Model file for the job. Use its own axes, mm. A direction names the side the tool comes from. Round coordinates to 2 decimals unless told otherwise and drop trailing zeros. Write each loop counter-clockwise with the first axis right and the second up, starting at its lowest first coordinate (ties: lowest second). Pieces come first, ordered by that corner, then holes. Notation, with made-up numbers: (-24, 53.5) - (12, 53.5) arc R7 ccw to (12, 66.5) - close; hole circle Ø7 at (20, -9). An arc over 180 degrees is marked (long way). One line per item, written item: value.
from build123d import *

# Parameters (mm, degrees)
BOSS_EXTRUDE1_DEPTH = 350


with BuildPart() as part:
    # Sketch1 → Boss-Extrude1 (new body)
    with BuildSketch(Plane.XY):
        with BuildLine():
            Line((0, 0), (30, 0))
            Line((30, 0), (30, 1))
            ThreePointArc((30, 1), (29.414213562, 2.414213562), (28, 3))
            Line((28, 3), (5, 3))
            ThreePointArc((5, 3), (3.585786438, 3.585786438), (3, 5))
            Line((3, 5), (3, 28))
            ThreePointArc((3, 28), (2.414213562, 29.414213562), (1, 30))
            Line((1, 30), (0, 30))
            Line((0, 30), (0, 0))
        make_face()
    extrude(amount=BOSS_EXTRUDE1_DEPTH)


solid = part.part
1. Drop flat-ended pins along their axis: pin 1 (12 mm diameter, centred on y = 23, z = 100, fed in from +X); pin 2 (12 mm diameter, centred on x = 10, z = 165, fed in from -Y); pin 3 (3 mm diameter, centred on y = 3, z = 238.5, fed in from +X); pin 4 (7 mm diameter, centred on x = 12, z = 141, fed in from +Y). Give the stop position or say it passes through.
Report:
pin 1: x = 3
pin 2: y = 0
pin 3: x = 29.94
pin 4: y = 3
2. Wall check: probe 1 along X at (y, z) = (14, 96); probe 2 along Y at (x, z) = (4.5, 296.5). Give the ranges that are in metal, low to high. Write a range as [from, to].
Report:
probe 1: [0, 3]
probe 2: [0, 3.06]
3. Band-saw the part on A-A on z = 243.5. Write the cut outline in (x, y).
Report:
outline: (0, 0) - (30, 0) - (30, 1) arc R2 ccw to (28, 3) - (5, 3) arc R2 cw to (3, 5) - (3, 28) arc R2 ccw to (1, 30) - (0, 30) - close
4. Band-saw the part on B-B on y = 15. Write the cut outline in (x, z).
Report:
outline: (0, 0) - (3, 0) - (3, 350) - (0, 350) - close
5. Tool access for faces 1 (the face through (17, 3, 173)), 2 (the face through (2.7, 9.5, 0)): list every direction of +Z, -Z, +X, -X, +Y, -Y with a clear straight run to the whole face (end or side of a thin tool).
Report:
face 1: +Z, -Z, +X, +Y
face 2: -Z, +X, -X, +Y, -Y
